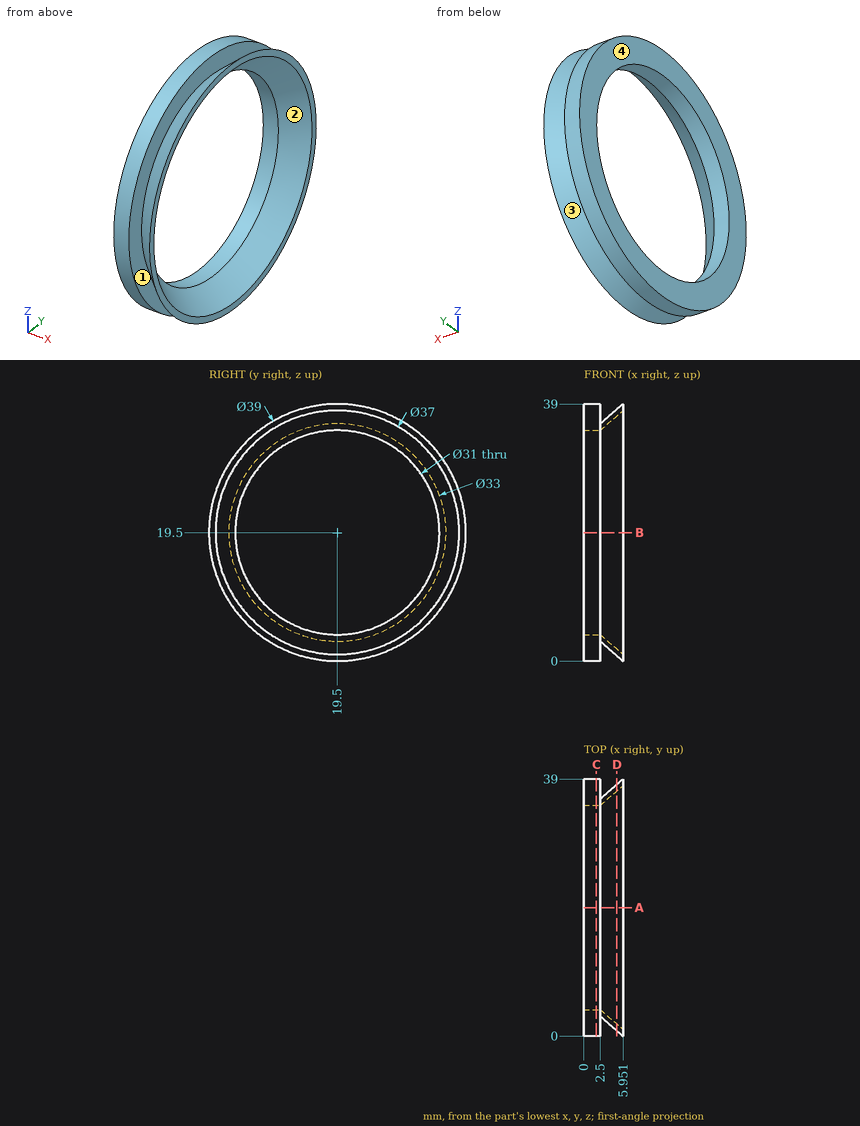
Job drawing, mm, ordinate dimensions from the low corner. One solid piece. A direction names the side the tool comes from. Coordinates: 2 decimals unless noted, no trailing zeros. Order: outer loops, then holes, each group sorted by start corner. A loop starts at its lowest first (then second) coordinate and runs counter-clockwise, first axis right, second up. Notation, with made-up numbers: M -8.5,40 L 49.5,40 A36 ccw 49.5,79 Z; hole C -17,-6 d6. An arc over 180 degrees is marked long. Return JSON: item names as keys, results as strings.
1. Tool access for the marked faces 3 and 4: list every direction of +Z, -Z, +X, -X, +Y, -Y with a clear straight run to the whole face (end or side of a thin tool).
Ans:
{"face 3": "none", "face 4": "+Z, -Z, -X, +Y, -Y"}
2. Saw through at D-D (x = 5). Give the cut face in (y, z).
Ans:
{"outline": "C 19.5,19.5 d37.35; hole C 19.5,19.5 d35.35"}
3. Drill centre lines: probe 1 along Y at (x, z) = (1.8, 19.5); probe 2 along Y at (x, z) = (0.4, 22). Where is each one in solid material? Low to high.
Ans:
{"probe 1": "0 to 4, 35 to 39", "probe 2": "0.16 to 4.2, 34.8 to 38.84"}
4. Pull direction Z, two halves, no side cores. Call the marked faces 1 and 2: +Z half, -Z half, draft (parallel to the pull), parting line (faces both ways), or undercut.
Ans:
{"face 1": "draft", "face 2": "undercut"}
5. Saw through at C-C (x = 1.9). Give the cut face in (y, z), and give its area (3 significant figures).
Ans:
{"outline": "C 19.5,19.5 d39; hole C 19.5,19.5 d31", "area": "440 mm^2"}
6. Flat gauge pins, fed straight in: pin 1 (1.5 mm diameter, centred on y = 27, z = 34, fed in from +X); pin 2 (1.5 mm diameter, centred on x = 4.5, z = 30.5, fed in from +Y) (1 decimal); pin 3 (12 mm diameter, centred on y = 4.5, z = 27, fed in from -X); pin 4 (1.5 mm diameter, centred on x = 5, y = 30, fed in from +Z). Where does each tip first touch, or does it go through?
Ans:
{"pin 1": "x = 4.31", "pin 2": "y = 35", "pin 3": "x = 0", "pin 4": "z = 35.86"}
7. Saw through at A-A (y = 19.5). Give the cut face in (x, z).
Ans:
{"outline": "M 0,0 L 2.5,0 L 2.5,3 L 5.95,0 L 5.95,1 L 2.5,4 L 0,4 Z; M 0,35 L 2.5,35 L 5.95,38 L 5.95,39 L 2.5,36 L 2.5,39 L 0,39 Z"}
